from build123d import *

# Parameters (mm, degrees)
M5_TAPPED_HOLE1_D     = 4.2
M5_TAPPED_HOLE1_DEPTH = 30
M5_TAPPED_HOLE1_TIP   = 1.2618073
CHAMFER1_SIZE         = 2


with BuildPart() as part:
    # Sketch1 → Revolve2 (revolve)
    with BuildSketch(Plane.XY, mode=Mode.PRIVATE) as revolve2_sk:
        with BuildLine():
            Line((-22, 63), (-22, 15))
            Line((-22, 15), (-27.5, 15))
            Line((-27.5, 15), (-27.5, 0))
            Line((-27.5, 0), (-17.5, 0))
            Line((-17.5, 0), (-17.5, 20))
            Line((-17.5, 20), (-17, 20))
            Line((-17, 20), (-17, 63))
            ThreePointArc((-17, 63), (-12.02081528, 75.02081528), (0, 80))
            Line((0, 80), (0, 85))
            ThreePointArc((0, 85), (-15.556349186, 78.556349186), (-22, 63))
        make_face()
    revolve(revolve2_sk.sketch.rotate(Axis((0, 0, 0), (0, 1, 0)), 270), axis=Axis((0, 0, 0), (0, 1, 0)))

    # M5 Tapped Hole1
    with Locations(Plane(origin=(-0.002180136, 7.524181673, 27.499999914), x_dir=(0.999999996858, 0, 7.9277686e-05), z_dir=(-7.9277686e-05, 0, 0.999999996858))):
        with Locations((0, 0)):
            Hole(M5_TAPPED_HOLE1_D / 2, depth=M5_TAPPED_HOLE1_DEPTH)
            with Locations((0, 0, -(M5_TAPPED_HOLE1_DEPTH + M5_TAPPED_HOLE1_TIP / 2))):  # 118° drill point
                Cone(0, M5_TAPPED_HOLE1_D / 2, M5_TAPPED_HOLE1_TIP, mode=Mode.SUBTRACT)

    # Chamfer1
    chamfer1_edges = [part.edges().sort_by_distance(p)[0] for p in [
        (0, 0, 17.5),
    ]]
    chamfer(chamfer1_edges, length=CHAMFER1_SIZE)


solid = part.part
Input: part model. Units: mm. Frame: model coordinates. A direction names the side the tool comes from. Coordinates: 2 decimals unless noted, no trailing zeros. Loops run counter-clockwise (first coordinate to the right, second up) from the corner with the lowest first, then second, coordinate; pieces in that order, holes last. Notation, with made-up numbers: (32.5, 70) - (65.5, 70) arc R11 ccw to (65.5, 77) - close; hole circle Ø3 at (65.25, -17.75). An arc over 180 degrees is marked (long way). Answer in a Markdown table with one row per item. Add a question column.
Item 1: Access query for faces 5 (the flat face through (-19, 0, -6)), 6 (the cylindrical face through (-16.855, 41.801, 2.213)), 7 (the cylindrical face through (21.477, 38.664, 4.769)). Directions: +Z, -Z, +X, -X, +Y, -Y. A direction counts if a zero-diameter tool reaches every point of the face in a straight line with its end or side. Return the directions, or none.
Item 2: Line query: line 1 along X through (y, z) = (14.25, 0); line 2 along Z through (x, y) = (5.5, 22.5); line 3 along X through (y, z) = (59.5, 4). Output: solid intervals per line, ascending. Write a range as [from, to].
Item 3: Mould query, pull axis Z, two halves, no side actions, for faces 1 (the cylindrical face through (-5.26, 11.13, -16.69)), 2 (the cylindrical face through (10.533, 7.395, -25.403)), 3 (the flat face through (-17, 20, 3)), 4 (the flat face through (-18.5, 15, -12.4)). Classes: released by +Z, released by -Z, zero draft, split by the parting line, or undercut.
Item 4: Section query B-B on y = 50. Return the cut outline in (x, z).
Item 5: Section query A-A on z = 0. Return the cut outline in (x, y).
Item 6: Contact query for flat-ended pins moving along their axis: P1, Ø1, axis at y = 32, z = -19, coming from the -X side; P2, Ø6, axis at x = -6, y = 28, coming from the -Z side; P3, Ø6, axis at x = -1, z = 5.5, coming from the -Y side. Output: stop coordinate, or through.
Recorded:
| question | item | result |
|---|---|---|
| 1 | face 5 | +Z, -Z, +X, -X, -Y |
| 1 | face 6 | -Y |
| 1 | face 7 | +Y |
| 2 | line 1 | [-27.5, -17.5], [17.5, 27.5] |
| 2 | line 2 | [-21.3, -16.09], [16.09, 21.3] |
| 2 | line 3 | [-21.63, -16.52], [16.52, 21.63] |
| 3 | face 1 | undercut |
| 3 | face 2 | split by the parting line |
| 3 | face 3 | undercut |
| 3 | face 4 | zero draft |
| 4 | outline | circle Ø44 at (0, 0); hole circle Ø34 at (0, 0) |
| 5 | outline | (-27.5, 0) - (-19.5, 0) - (-17.5, 2) - (-17.5, 20) - (-17, 20) - (-17, 63) arc R17 cw to (17, 63) - (17, 20) - (17.5, 20) - (17.5, 2) - (19.5, 0) - (27.5, 0) - (27.5, 15) - (22, 15) - (22, 63) arc R22 ccw to (-22, 63) - (-22, 15) - (-27.5, 15) - close |
| 6 | P1 | x = -11.91 |
| 6 | P2 | z = -21.79 |
| 6 | P3 | y = 77.67 |
